Here's how the part is built. I have some questions about the finished solid (model axes, mm). A direction names the side the tool comes from. Coordinates: 2 decimals unless noted, no trailing zeros. Loops run counter-clockwise (first coordinate to the right, second up) from the corner with the lowest first, then second, coordinate; pieces in that order, holes last.
```python
from build123d import *

# Parameters (mm, degrees)
SKETCH2_R           = 89.5
BOSS_EXTRUDE1_DEPTH = 37
SHELL1_T            = -3


with BuildPart() as part:
    # Sketch1 → Revolve1 (revolve)
    with BuildSketch(Plane.XY, mode=Mode.PRIVATE) as revolve1_sk:
        Polygon((0, 0), (125, 0), (125, 185), (91.5, 185), (91.5, 270), (75, 270), (75, 290), (0, 290), align=None)
    revolve(revolve1_sk.sketch.rotate(Axis((0, 290, 0), (0, -1, 0)), 90), axis=Axis((0, 290, 0), (0, -1, 0)))

    # Sketch2 → Boss-Extrude1 (add)
    with BuildSketch(Plane.XZ):
        with Locations(Location((17, 0, 0), (0, 0, 90))):
            Circle(SKETCH2_R)
    extrude(amount=BOSS_EXTRUDE1_DEPTH)

    # Shell1
    shell1_openings = [part.faces().sort_by_distance(p)[0] for p in [
        (17, -37, 0),
        (0, 290, 0),
    ]]
    offset(amount=SHELL1_T, openings=shell1_openings, kind=Kind.INTERSECTION)


solid = part.part
```
1. I want a section at D-D (y = 246.5). Please give me the cut outline in (x, z).
2. On a 3-axis mill with a long thin cutter (end or side, diameter ignored), from which of +Z, -Z, +X, -X, +Y, -Y can I reach the whole of each face in a straight line? I mean faces 1 (the cylindrical face through (-9.88, -18.24, 85.37)), 2 (the cylindrical face through (119.1, 93.75, -26.45)), 3 (the flat face through (-75, 270, -7)), 4 (the flat face through (-28, 290, -67)), 5 (the cylindrical face through (-5.5, 93.8, -124.88)). Say none if no direction works.
3. For pin 1 (3 mm diameter, centred on y = 205, z = -69.5, fed in from -X); pin 2 (10 mm diameter, centred on y = 61, z = 37.5, fed in from +X); pin 3 (2 mm diameter, centred on x = -71.5, z = -89, fed in from +Y), each with a flat end and sliding along its axis, tell me the tip position at first contact or that it passes through.
4. We'd pull the mould along X, two halves only. Please class faces 6 (the flat face through (-57, 0, -54)), 7 (the cylindrical face through (78.515, 225.095, 40.837)), 8 (the cylindrical face through (-27.484, 228.095, 87.275)): +X half, -X half, draft (parallel to the pull), parting line (faces both ways), or undercut.
5. I want a section at C-C (z = -97). Please give me the cut outline in (x, y).
6. I need wall thicknesses on line 1 along Y through (x, z) = (-101.5, -22.5); line 2 along X through (y, z) = (-22, 0); line 3 along Y through (x, z) = (-88.5, -11). Which ranges of each line are inside material? Lowest first, please.
Response values:
1. outline: circle Ø183 at (0, 0); hole circle Ø177 at (0, 0)
2. face 1: -Y
2. face 2: none
2. face 3: +Y
2. face 4: +Z, -Z, +X, -X, +Y
2. face 5: +Y, -Y
3. pin 1: stops at x = -61.22
3. pin 2: stops at x = 120.7
3. pin 3: stops at y = 185
4. face 6: draft
4. face 7: undercut
4. face 8: parting line
5. outline: (-78.84, 0) - (78.84, 0) - (78.84, 185) - (-78.84, 185) - close; hole (-73.99, 3) - (73.99, 3) - (73.99, 182) - (-73.99, 182) - close
6. line 1: y = 0 to 3, 182 to 185
6. line 2: x = -72.5 to -69.5, 103.5 to 106.5
6. line 3: y = 0 to 3, 182 to 270
